```python
from build123d import *

# Parameters (mm, degrees)
SKETCH_1_W                  = 153.5
SKETCH_1_H                  = 80
EXTRUDE_1_DEPTH             = 7.5
HOLE_WIZARD_25_0_25_1_D     = 25
HOLE_WIZARD_M8_1_AT_2_COUNT = 2
HOLE_WIZARD_M8_1_AT_2_PITCH = 60
SKETCH_6_R                  = 56
CUT_EXTRUDE_1_DEPTH         = 10
CHAMFER_1_SIZE              = 2


with BuildPart() as part:
    # 草图1 → 凸台-拉伸1 (new, symmetric)
    with BuildSketch(Plane.XY):
        Rectangle(SKETCH_1_W, SKETCH_1_H)
    extrude(amount=EXTRUDE_1_DEPTH, both=True)

    # Ø25.0 (25) 直径孔1 (through all)
    with Locations(Plane.XY.offset(7.5)):
        with Locations((36.75, 0)):
            Hole(HOLE_WIZARD_25_0_25_1_D / 2)

    # 草图4 → M8 螺纹孔1 (revolve, cut)
    with BuildSketch(Plane(origin=(76.75, -30, 0), x_dir=(0, 0, -1), z_dir=(0, 1, 0))):
        Polygon((0, 0), (0, 21.792926105), (3.4, 19.75), (3.4, 0), align=None)
    hole_wizard_m8_1 = revolve(axis=Axis((83.1, -30, 0), (-1, 0, 0)), mode=Mode.SUBTRACT)

    # M8 螺纹孔1 at 2: M8 螺纹孔1 ×2
    with Locations(*[(0, i * HOLE_WIZARD_M8_1_AT_2_PITCH, 0) for i in range(1, HOLE_WIZARD_M8_1_AT_2_COUNT)]):
        add(hole_wizard_m8_1, mode=Mode.SUBTRACT)

    # 镜向1: M8 螺纹孔1 across plane
    add(hole_wizard_m8_1.mirror(Plane(origin=(0, 0, 0), x_dir=(0, 0, 1), z_dir=(1, 0, 0))), mode=Mode.SUBTRACT)

    # 镜向1 copy 1 sketch → 镜向1 copy 1 (revolve, cut)
    with BuildSketch(Plane(origin=(-76.75, 30, 0), x_dir=(0, 0, -1), z_dir=(0, 1, 0))):
        Polygon((0, 0), (0, -21.792926105), (3.4, -19.75), (3.4, 0), align=None)
    revolve(axis=Axis((-83.1, 30, 0), (-1, 0, 0)), mode=Mode.SUBTRACT)

    # 草图6 → 切除-拉伸1 (cut)
    with BuildSketch(Plane.ZY.offset(76.75)):
        with Locations((-52.5, 0)):
            Circle(SKETCH_6_R)
    extrude(amount=-CUT_EXTRUDE_1_DEPTH, mode=Mode.SUBTRACT)

    # 倒角1
    chamfer_1_edges = [part.edges().sort_by_distance(p)[0] for p in [
        (76.75, -40, 0),
        (-76.75, -40, 0),
        (-76.75, 40, 0),
        (76.75, 40, 0),
    ]]
    chamfer(chamfer_1_edges, length=CHAMFER_1_SIZE)


solid = part.part
```
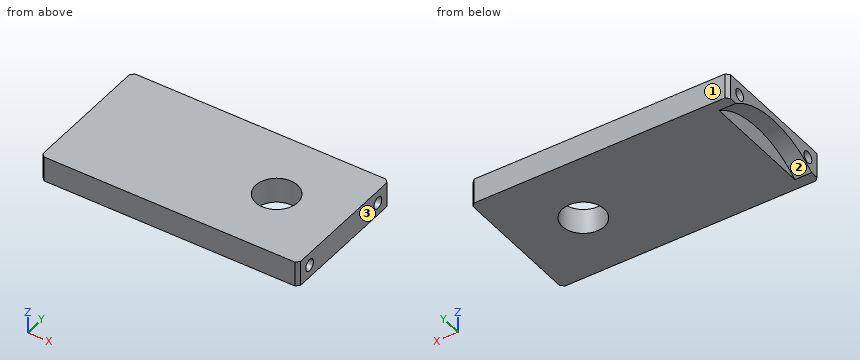
Check sheet for the modelled part. Datum: model origin and axes. Units: mm. Face numbers are marked on the shaded views. Round coordinates to 2 decimals unless told otherwise and drop trailing zeros. Loops run counter-clockwise (first coordinate to the right, second up) from the corner with the lowest first, then second, coordinate; pieces in that order, holes last. Notation, with made-up numbers: (48.25, 36) -> (65.25, 36) arc R25 ccw to (65.25, 72) -> close; hole circle Ø8 at (78, -1.5). An arc over 180 degrees is marked (long way). Write item = value, one per line. Start each with the question number.
1) Sectioned sample at D-D, the plane y = -14.5. Record the cut outline in (x, z).
2) Sectioned sample at A-A, the plane y = 0. Record the cut outline in (x, z), plus the area to 3 significant figures.
3) Sectioned sample at C-C, the plane x = 36.75. Record the cut outline in (y, z), plus the area to 3 significant figures.
4) Sectioned sample at B-B, the plane z = 5.25. Record the cut outline in (x, y), plus the area to 3 significant figures.
5) Gauge pin test, flat ends, axial feed: pin 1 Ø5.5 at (y, z) = (9.5, -3.5) entering from -X; pin 2 Ø5.5 at (y, z) = (-30, 0) entering from -X. Record the tip position at first contact, or that the pin passes through.
6) Thickness scan on probe 1 along Y at (x, z) = (63, 0); probe 2 along Y at (x, z) = (36.75, 4.5); probe 3 along Y at (x, z) = (-58.5, -1.5). Record the ranges inside material, lowest first.
7) Release check for a two-part mould opening along Y. For the marked faces 1, 2 and 3 record: released by +Y, released by -Y, zero draft, split by the parting line, or undercut.
Results are:
q1.outline = (-76.75, 1.59) -> (-66.75, 1.59) -> (-66.75, -7.5) -> (76.75, -7.5) -> (76.75, 7.5) -> (-76.75, 7.5) -> close
q2.outline = (-76.75, 3.5) -> (-66.75, 3.5) -> (-66.75, -7.5) -> (24.25, -7.5) -> (24.25, 7.5) -> (-76.75, 7.5) -> close; (49.25, -7.5) -> (76.75, -7.5) -> (76.75, 7.5) -> (49.25, 7.5) -> close
q2.area = 1,820 mm^2
q3.outline = (-40, -7.5) -> (-12.5, -7.5) -> (-12.5, 7.5) -> (-40, 7.5) -> close; (12.5, -7.5) -> (40, -7.5) -> (40, 7.5) -> (12.5, 7.5) -> close
q3.area = 825 mm^2
q4.outline = (-76.75, -38) -> (-74.75, -40) -> (74.75, -40) -> (76.75, -38) -> (76.75, 38) -> (74.75, 40) -> (-74.75, 40) -> (-76.75, 38) -> close; hole circle Ø25 at (36.75, 0)
q4.area = 11,800 mm^2
q5.pin_1 = -66.75
q5.pin_2 = -56.61
q6.probe_1 = -40 to -33.4, -26.6 to 26.6, 33.4 to 40
q6.probe_2 = -40 to -12.5, 12.5 to 40
q6.probe_3 = -40 to -33.05, -26.95 to 26.95, 33.05 to 40
q7.face_1 = released by +Y
q7.face_2 = undercut
q7.face_3 = zero draft
